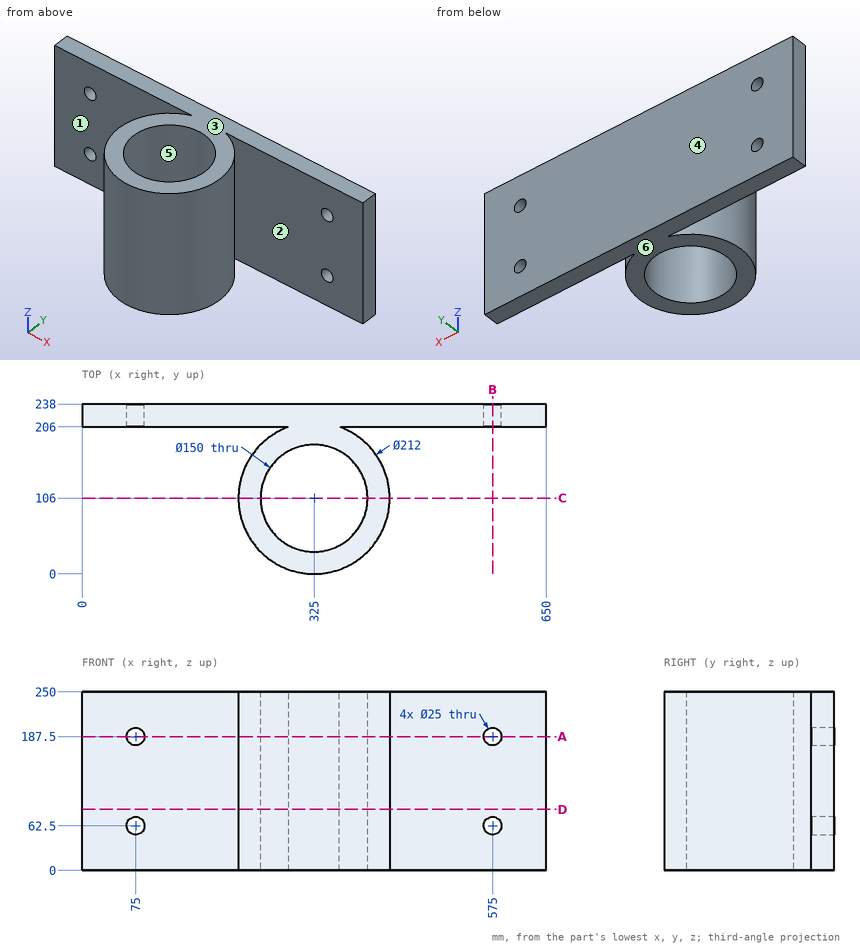
Print and shaded views of the part. All mm, measured from the part's lowest x, y and z. A direction names the side the tool comes from. Coordinates: 2 decimals unless noted, no trailing zeros. Order: outer loops, then holes, each group sorted by start corner. A loop starts at its lowest first (then second) coordinate and runs counter-clockwise, first axis right, second up. Notation, with made-up numbers: (62.5, 63.5) - (84.5, 63.5) arc R13 ccw to (84.5, 84.5) - close; hole circle Ø1 at (76, 72.25). An arc over 180 degrees is marked (long way). Return JSON: item names as keys, results as strings. Group by question number.
Item 1: Cut at D-D (z = 85.5). List the corners of the cut face in (x, y).
Item 2: Drill centre lines: probe 1 along X at (y, z) = (225, 62); probe 2 along Y at (x, z) = (325, 122); probe 3 along Y at (x, z) = (464.5, 56). Where is each one in solid material? Low to high. Write a range as from..to.
Item 3: Cut at A-A (z = 187.5). List the corners of the cut face in (x, y).
Item 4: Cut at B-B (x = 575). List the corners of the cut face in (y, z).
Item 5: Pin check, flat tips, straight feed: pin 1 (20 mm diameter, centred on x = 575, z = 62.5, fed in from +Y); pin 2 (2 mm diameter, centred on y = 132.5, z = 103.5, fed in from +X); pin 3 (12 mm diameter, centred on x = 190.5, z = 104.5, fed in from -Y); pin 4 (4 mm diameter, centred on y = 74.5, z = 206, fed in from +X). Stop position of each tip, or through.
Item 6: Pull direction Y, two halves, no side cores. Call the marked faces 4, 5 and 6: pulls with the +Y half, pulls with the -Y half, needs draft (parallel to the pull), parting line crosses it, or undercut.
Item 7: Which spindle directions (+Z, -Z, +X, -X, +Y, -Y) get a long thin tool onto all of the face, cutting with end or side? Do the marked faces 1, 2 and 3. Say none if no direction does.
Item 8: Cut at C-C (y = 106). List the corners of the cut face in (x, z).
Check values:
{
 "1": {"outline": "(0, 206) - (289.84, 206) arc R106 ccw (long way) to (360.16, 206) - (650, 206) - (650, 238) - (0, 238) - close; hole circle Ø150 at (325, 106)"},
 "2": {"probe 1": "x = 0..62.51, 87.49..562.51, 587.49..650", "probe 2": "y = 0..31, 181..238", "probe 3": "y = 206..238"},
 "3": {"outline": "(0, 206) - (62.5, 206) - (62.5, 238) - (0, 238) - close; (87.5, 206) - (289.84, 206) arc R106 ccw (long way) to (360.16, 206) - (562.5, 206) - (562.5, 238) - (87.5, 238) - close; (587.5, 206) - (650, 206) - (650, 238) - (587.5, 238) - close; hole circle Ø150 at (325, 106)"},
 "4": {"outline": "(206, 0) - (238, 0) - (238, 50) - (206, 50) - close; (206, 75) - (238, 75) - (238, 175) - (206, 175) - close; (206, 200) - (238, 200) - (238, 250) - (206, 250) - close"},
 "5": {"pin 1": "passes through", "pin 2": "stops at x = 427.89", "pin 3": "stops at y = 206", "pin 4": "stops at x = 426.81"},
 "6": {"face 4": "pulls with the +Y half", "face 5": "undercut", "face 6": "needs draft"},
 "7": {"face 1": "+Z, -Z, -X", "face 2": "+Z, -Z, +X", "face 3": "+Z, +X, -X, +Y, -Y"},
 "8": {"outline": "(219, 0) - (250, 0) - (250, 250) - (219, 250) - close; (400, 0) - (431, 0) - (431, 250) - (400, 250) - close"}
}
